from build123d import *

# Parameters (mm, degrees)
SKETCH2_R          = 11
SKETCH2_R_2        = 2.5
CUT_EXTRUDE1_DEPTH = 10
FILLET1_R          = 3
FILLET2_R          = 1


with BuildPart() as part:
    # Sketch1 → Revolve1 (revolve)
    with BuildSketch(Plane.XY, mode=Mode.PRIVATE) as revolve1_sk:
        Polygon((-61.497364751, 54.207400123), (-61.497364751, 63.064837562), (-60.157873326, 63.064837562), (-60.157873326, 60.798367254), (-54.997364751, 60.798367254), (-54.997364751, 55.593672907), (-41.497364751, 54.299979424), (-41.497364751, 25.564837562), (-43.497364751, 25.564837562), (-43.497364751, 52.482475479), align=None)
    revolve(revolve1_sk.sketch.rotate(Axis((-61.497364751, 25.564837562, 0), (1, 0, 0)), 90), axis=Axis((-61.497364751, 25.564837562, 0), (1, 0, 0)))

    # Sketch2 → Cut-Extrude1 (cut)
    with BuildSketch(Plane(origin=(-41.497364751, 0, 0), x_dir=(0, 0, -1), z_dir=(1, 0, 0))):
        with Locations((0, 25.564837562)):
            Circle(SKETCH2_R)
        with Locations((-14.598664639, 41.420145509)):
            Circle(SKETCH2_R_2)
        with Locations((14.598664639, 41.420145509)):
            Circle(SKETCH2_R_2)
        with Locations((14.598664639, 9.709529615)):
            Circle(SKETCH2_R_2)
        with Locations((-14.598664639, 9.709529615)):
            Circle(SKETCH2_R_2)
    extrude(amount=-CUT_EXTRUDE1_DEPTH, mode=Mode.SUBTRACT)

    # Fillet1
    fillet1_edges = [part.edges().sort_by_distance(p)[0] for p in [
        (-41.497364751, 25.564837562, -28.735141862),
    ]]
    fillet(fillet1_edges, radius=FILLET1_R)

    # Fillet2
    fillet2_edges = [part.edges().sort_by_distance(p)[0] for p in [
        (-54.997364751, 25.564837562, -35.233529691),
    ]]
    fillet(fillet2_edges, radius=FILLET2_R)


solid = part.part
Geometry check sheet. Reference: the model listing, model coordinates, mm. A direction names the side the tool comes from. Round coordinates to 2 decimals unless told otherwise and drop trailing zeros. Write each loop counter-clockwise with the first axis right and the second up, starting at its lowest first coordinate (ties: lowest second). Pieces come first, ordered by that corner, then holes.
Item 1: Section check D-D (x = -48). Record the boundary of the cut face in (y, z), plus the area to 3 significant figures.
Determined:
outline: circle Ø58.72 at (25.56, 0); hole circle Ø54.7 at (25.56, 0)
area: 358 mm2
Item 2: Section check C-C (y = 11). Give the number of separate pieces and of enclosed holes in the cut face, plus the area to 3 significant figures.
Determined:
separate pieces: 3
enclosed holes: 0
area: 240 mm2
Item 3: Section check A-A (z = 0). Record the boundary of the cut face in (x, y), plus the area to 3 significant figures.
Determined:
outline: (-61.5, -11.94) - (-60.16, -11.94) - (-60.16, -9.67) - (-56, -9.67) arc R1 ccw to (-55, -8.67) - (-55, -4.46) - (-44.21, -3.43) arc R3 ccw to (-41.5, -0.44) - (-41.5, 14.56) - (-43.5, 14.56) - (-43.5, -1.35) - (-61.5, -3.08) - close; (-61.5, 54.21) - (-43.5, 52.48) - (-43.5, 36.56) - (-41.5, 36.56) - (-41.5, 51.57) arc R3 ccw to (-44.21, 54.56) - (-55, 55.59) - (-55, 59.8) arc R1 ccw to (-56, 60.8) - (-60.16, 60.8) - (-60.16, 63.06) - (-61.5, 63.06) - close
area: 210 mm2
Item 4: Section check B-B (x = -59.25). Record the boundary of the cut face in (y, z).
Determined:
outline: circle Ø70.47 at (25.56, 0); hole circle Ø56.85 at (25.56, 0)
Item 5: Go/stop test with flat-tipped pins: pin 1 Ø8 at (y, z) = (45, -5.5) entering from -X; pin 2 Ø5 at (x, z) = (-58.5, 19) entering from -Y; pin 3 Ø1 at (y, z) = (-1.5, -1) entering from +X. Record where each tip stops, or that it passes through.
Determined:
pin 1: stops at x = -43.5
pin 2: stops at y = -7.79
pin 3: stops at x = -41.55
Item 6: Access from +Z, -Z, +X, -X, +Y, -Y to the whole of each face (thin tool, end or side, straight path). Record for faces 1 (the face through (-60.158, 37, -34)), 2 (the face through (-42.483, 43.528, 13.255)).
Determined:
face 1: +X
face 2: +X, -X
Item 7: Material ranges on line 1 along X through (y, z) = (14, 30); line 2 along X through (y, z) = (38, -11); line 3 along Y through (x, z) = (-54.25, -10), recorded low to high.
Determined:
line 1: x = -61.5 to -55
line 2: x = -43.5 to -41.5
line 3: y = -2.67 to -0.53, 51.66 to 53.8
Item 8: Mould release check, pull along Z, two halves, no side actions. Record for faces 3 (the face through (-61.497, 53, 9)), 4 (the face through (-43.497, 37, 0)), 5 (the face through (-47.132, 16.771, 27.923)): +Z half, -Z half, draft (parallel to the pull), parting line (faces both ways), or undercut.
Determined:
face 3: draft
face 4: undercut
face 5: parting line
